Study the drawing (mm; zero at the part's minimum x, y, z) and answer. Round coordinates to 2 decimals unless told otherwise and drop trailing zeros. Order: outer loops, then holes, each group sorted by start corner. A loop starts at its lowest first (then second) coordinate and runs counter-clockwise, first axis right, second up. Notation, with made-up numbers: (37.25, 86.5) - (42.25, 86.5) arc R29 cw to (42.25, 106.5) - close; hole circle Ø3 at (6, -20.5). An arc over 180 degrees is marked (long way). Put each result on its own line as item: value. Start each with the question number.
Q1. Section B-B on y = 65 is taken. Give the vertices of the cut face in (x, z).
Q2. Section D-D on x = 58.5 is taken. Give the vertices of the cut face in (y, z), then the cut area to 3 significant figures.
Q3. Find the intervals of material crossed by line 1 along Y through (x, z) = (240, 8); line 2 along Y through (x, z) = (31, 12.25); line 3 along X through (y, z) = (106, 6.25), in increasing order. Write a range as from..to.
Q4. Section C-C on z = 5 is taken. Give the vertices of the cut face in (x, y).
Q5. Section A-A on x = 440 is taken. Give the vertices of the cut face in (y, z), then the cut area to 3 significant figures.
Q6. Each of these flat-tipped pins is pushed along its axis until it touches: pin 1 Ø1 at (x, z) = (348, 9.5) entering from -Y; pin 2 Ø4 at (x, z) = (563.5, 5.5) entering from +Y. Where does it stop, or does it pass through?
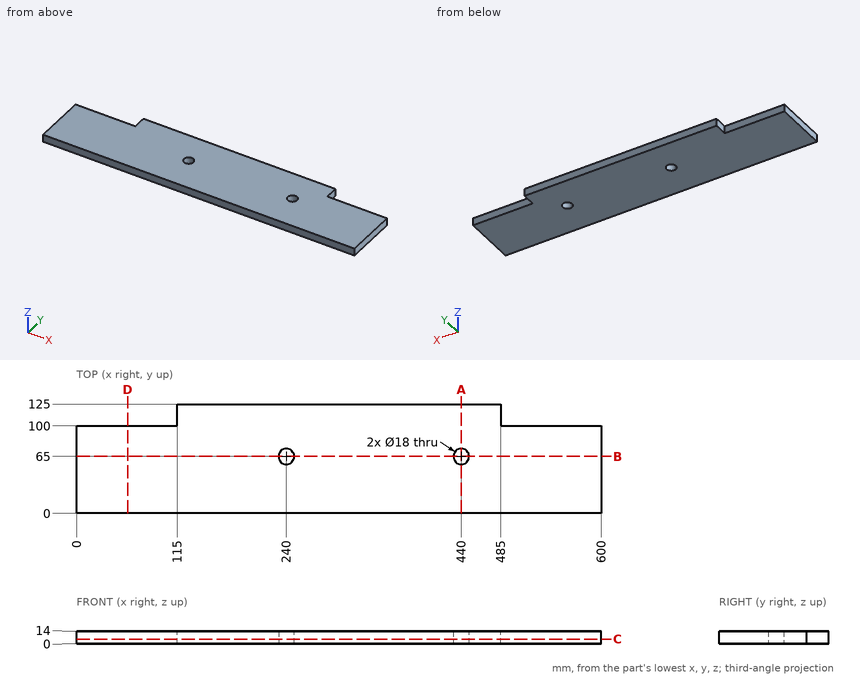
Findings:
1. outline: (0, 0) - (231, 0) - (231, 14) - (0, 14) - close; (249, 0) - (431, 0) - (431, 14) - (249, 14) - close; (449, 0) - (600, 0) - (600, 14) - (449, 14) - close
2. outline: (0, 0) - (100, 0) - (100, 14) - (0, 14) - close
2. area: 1,400 mm2
3. line 1: 0..56, 74..125
3. line 2: 0..100
3. line 3: 115..485
4. outline: (0, 0) - (600, 0) - (600, 100) - (485, 100) - (485, 125) - (115, 125) - (115, 100) - (0, 100) - close; hole circle Ø18 at (240, 65); hole circle Ø18 at (440, 65)
5. outline: (0, 0) - (56, 0) - (56, 14) - (0, 14) - close; (74, 0) - (125, 0) - (125, 14) - (74, 14) - close
5. area: 1,500 mm2
6. pin 1: y = 0
6. pin 2: y = 100
